Check sheet for the modelled part. Datum: model origin and axes. Units: mm. A direction names the side the tool comes from. Give positions to 0.01 mm unless a question says otherwise; leave off trailing zeros. Loops run counter-clockwise (first coordinate to the right, second up) from the corner with the lowest first, then second, coordinate; pieces in that order, holes last. Notation, with made-up numbers: M 78.5,-10.5 L 110.5,-10.5 A21 cw 110.5,27.5 Z; hole C 18,37 d9. An arc over 180 degrees is marked long. One line per question, with ' | ' between items. Start each with the question number.
from build123d import *

# Parameters (mm, degrees)
BOSS_EXTRUDE1_DEPTH = 45
SKETCH2_R           = 8
CUT_EXTRUDE1_DEPTH  = 84.024092889


with BuildPart() as part:
    # Sketch1 → Boss-Extrude1 (new body)
    with BuildSketch(Plane.XY):
        with BuildLine():
            Line((0, 0), (0, -57))
            ThreePointArc((0, -57), (1.464466094, -60.535533906), (5, -62))
            Line((5, -62), (27, -62))
            ThreePointArc((27, -62), (30.535533906, -60.535533906), (32, -57))
            Line((32, -57), (32, 0))
            Line((32, 0), (29, 0))
            Line((29, 0), (29, -57))
            ThreePointArc((29, -57), (28.414213562, -58.414213562), (27, -59))
            Line((27, -59), (5, -59))
            ThreePointArc((5, -59), (3.585786438, -58.414213562), (3, -57))
            Line((3, -57), (3, 0))
            Line((3, 0), (0, 0))
        make_face()
    extrude(amount=BOSS_EXTRUDE1_DEPTH)

    # Sketch2 → Cut-Extrude1 (cut, through all)
    with BuildSketch(Plane(origin=(32, 0, 0), x_dir=(0, 0, -1), z_dir=(1, 0, 0))):
        with Locations((-22.5, -12)):
            Circle(SKETCH2_R)
    extrude(amount=-CUT_EXTRUDE1_DEPTH, mode=Mode.SUBTRACT)


solid = part.part
Q1. Cross-section at D-D (z = 16.5). Record the cut outline in (x, y).
Q2. Cross-section at C-C (y = -12). Record the cut outline in (x, z), and give its area (3 significant figures).
Q3. Material ranges on probe 1 along X at (y, z) = (-3, 42.5); probe 2 along Y at (x, z) = (17, 18.5); probe 3 along Y at (x, z) = (29.75, 22.5), recorded low to high. Write a range as from..to.
Q4. Cross-section at B-B (z = 22.5). Record the cut outline in (x, y), and give its area (3 significant figures).
Q5. Depth check by flat-ended pin: P1, Ø9.5, axis at y = -12, z = 22.5, coming from the -X side; P2, Ø10, axis at y = -8, z = 11.5, coming from the -X side; P3, Ø6.5, axis at x = 11, z = 32.5, coming from the +Y side; P4, Ø6, axis at x = 6.5, z = 23.5, coming from the +Y side. Enter the tip coordinate at first touch or a pass-through.
Q6. Draft check along X on faces 3 (the flat face through (2, -38, 45)), 4 (the cylindrical face through (1, -60, 22)), 5 (the flat face through (16, -59, 22)), 6 (the flat face through (3, -29, 22)). Enter one of: released by +X, released by -X, zero draft, split by the parting line, or undercut.
Q7. Access from +Z, -Z, +X, -X, +Y, -Y to the whole of each face (thin tool, end or side, straight path). Record for faces 1 (the cylindrical face through (28.43, -58.4, 22.18)), 2 (the cylindrical face through (30, -61, 22)).
Q8. Cross-section at A-A (y = -47.5). Record the cut outline in (x, z).
Solved:
1) outline: M 0,-57 A5 ccw 5,-62 L 27,-62 A5 ccw 32,-57 L 32,-17.29 L 29,-17.29 L 29,-57 A2 cw 27,-59 L 5,-59 A2 cw 3,-57 L 3,-17.29 L 0,-17.29 Z; M 0,-6.71 L 3,-6.71 L 3,0 L 0,0 Z; M 29,-6.71 L 32,-6.71 L 32,0 L 29,0 Z
2) outline: M 0,0 L 3,0 L 3,14.5 L 0,14.5 Z; M 0,30.5 L 3,30.5 L 3,45 L 0,45 Z; M 29,0 L 32,0 L 32,14.5 L 29,14.5 Z; M 29,30.5 L 32,30.5 L 32,45 L 29,45 Z | area: 174 mm²
3) probe 1: x = 0..3, 29..32 | probe 2: y = -62..-59 | probe 3: y = -61.18..-20, -4..0
4) outline: M 0,-57 A5 ccw 5,-62 L 27,-62 A5 ccw 32,-57 L 32,-20 L 29,-20 L 29,-57 A2 cw 27,-59 L 5,-59 A2 cw 3,-57 L 3,-20 L 0,-20 Z; M 0,-4 L 3,-4 L 3,0 L 0,0 Z; M 29,-4 L 32,-4 L 32,0 L 29,0 Z | area: 345 mm²
5) P1: passes through | P2: stops at x = 0 | P3: stops at y = -59 | P4: stops at y = -58.32
6) face 3: zero draft | face 4: released by -X | face 5: undercut | face 6: undercut
7) face 1: +Z, -Z, +Y | face 2: +Z, -Z, +X, -Y
8) outline: M 0,0 L 3,0 L 3,45 L 0,45 Z; M 29,0 L 32,0 L 32,45 L 29,45 Z
